Part model, mm, in its own coordinate system. Round coordinates to 2 decimals unless told otherwise and drop trailing zeros. Order: outer loops, then holes, each group sorted by start corner. A loop starts at its lowest first (then second) coordinate and runs counter-clockwise, first axis right, second up. Notation, with made-up numbers: (69, -7) -> (122, -7) arc R12 ccw to (122, 16) -> close; hole circle Ø10 at (-37, 22). An arc over 180 degrees is marked (long way). Use CSV: the item, a comma, the result in double quotes.
```python
from build123d import *

# Parameters (mm, degrees)
BOSS_EXTRUDE1_DEPTH = 1.6002
SKETCH2_R           = 1.5875
CUT_EXTRUDE1_DEPTH  = 1.6002


with BuildPart() as part:
    # Sketch1 → Boss-Extrude1 (new body)
    with BuildSketch(Plane.XY):
        with BuildLine():
            add(Edge.make_bspline(
                [(0, -28.1686), (-7.577848525, -28.285084622), (-14.719054348, -23.91013337), (-19.05, -17.8562)],
                knots=[0, 0, 0, 0, 1, 1, 1, 1], degree=3))
            ThreePointArc((-19.05, -17.8562), (-23.254686005, -9.371516124), (-24.6126, 0))
            ThreePointArc((-24.6126, 0), (-23.254686005, 9.371516124), (-19.05, 17.8562))
            add(Edge.make_bspline(
                [(0, 28.1686), (-7.577848525, 28.285084622), (-14.719054348, 23.91013337), (-19.05, 17.8562)],
                knots=[0, 0, 0, 0, 1, 1, 1, 1], degree=3))
            add(Edge.make_bspline(
                [(0, 28.1686), (7.577848525, 28.285084622), (14.719054348, 23.91013337), (19.05, 17.8562)],
                knots=[0, 0, 0, 0, 1, 1, 1, 1], degree=3))
            ThreePointArc((19.05, 17.8562), (23.254686005, 9.371516124), (24.6126, 0))
            ThreePointArc((24.6126, 0), (23.254686005, -9.371516124), (19.05, -17.8562))
            add(Edge.make_bspline(
                [(0, -28.1686), (7.577848525, -28.285084622), (14.719054348, -23.91013337), (19.05, -17.8562)],
                knots=[0, 0, 0, 0, 1, 1, 1, 1], degree=3))
        make_face()
    extrude(amount=BOSS_EXTRUDE1_DEPTH)

    # Sketch2 → Cut-Extrude1 (cut)
    with BuildSketch(Plane.XY.offset(1.6002)):
        with Locations((-12.7, 0)):
            Circle(SKETCH2_R)
        with Locations((12.7, 0)):
            Circle(SKETCH2_R)
    extrude(amount=-CUT_EXTRUDE1_DEPTH, mode=Mode.SUBTRACT)


solid = part.part
```
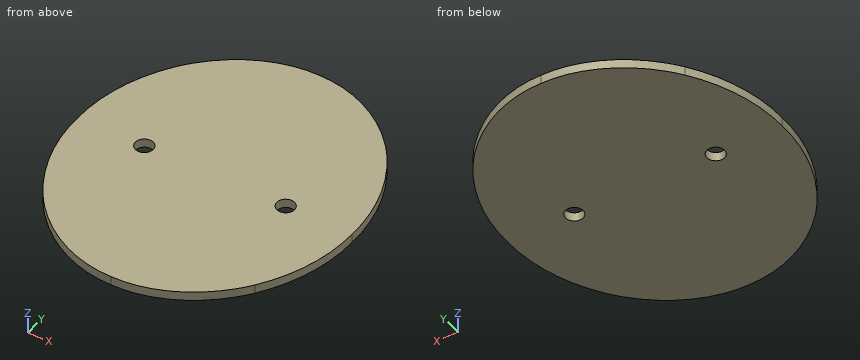
(1) Cut at B-B, the plane y = 15. Give the cut face in (x, z).
Reply:
outline,"(-20.85, 0) -> (20.85, 0) -> (20.85, 1.6) -> (-20.85, 1.6) -> close"
(2) Probe probe 1 along X at (y, z) = (0.5, 1.3); probe 2 along Y at (x, z) = (-12.7, 0.6); probe 3 along Y at (x, z) = (-13, 0.6). List the from-to ranges inside material, lowest first. Write a range as [from, to].
Reply:
probe 1,"[-24.62, -14.21], [-11.19, 11.19], [14.21, 24.62]"
probe 2,"[-24.1, -1.59], [1.59, 24.1]"
probe 3,"[-23.89, -1.56], [1.56, 23.89]"
(3) Cut at C-C, the plane y = 8.5. Give the cut face in (x, z), then the cut area to 3 significant figures.
Reply:
outline,"(-23.51, 0) -> (23.51, 0) -> (23.51, 1.6) -> (-23.51, 1.6) -> close"
area,"75.2 mm2"
(4) Cut at A-A, the plane z = 0.25. State how many separate pieces and enclosed holes the cut face has, then the cut area to 3 significant figures.
Reply:
separate pieces,"1"
enclosed holes,"2"
area,"2,160 mm2"
(5) Drop flat-ended pins along their axis: P1, Ø3.5, axis at x = -12.7, y = 0, coming from the -Z side; P2, Ø1.9, axis at x = 12.7, y = 0, coming from the +Z side. Give the stop position or say it passes through.
Reply:
P1,"z = 0"
P2,"through"
